Input: part model. Units: mm. Frame: model coordinates. Face numbers are marked on the shaded views. A direction names the side the tool comes from. Give positions to 0.01 mm unless a question says otherwise; leave off trailing zeros. Loops run counter-clockwise (first coordinate to the right, second up) from the corner with the lowest first, then second, coordinate; pieces in that order, holes last. Notation, with made-up numbers: (-34, -23.75) -> (3, -23.75) arc R6 ccw to (3, -15.75) -> close; hole circle Ø9 at (-29, -39). An arc over 180 degrees is marked (long way). Use CSV: the item, a comma, the result in double quotes.
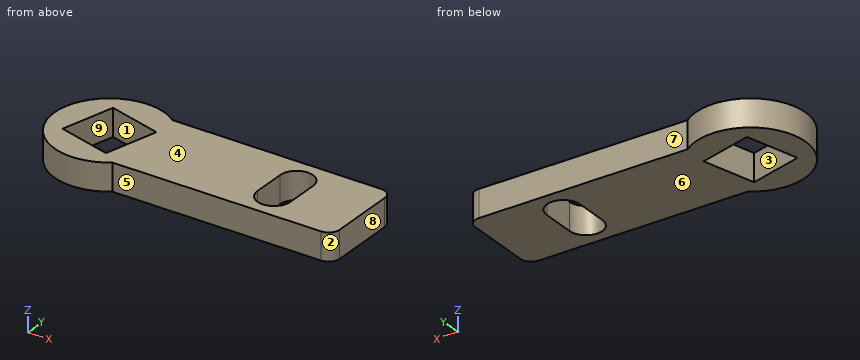
```python
from build123d import *

# Parameters (mm, degrees)
EXTRUDE_1_DEPTH     = 1.25
CUT_EXTRUDE_1_DEPTH = 24.669600757
FILLET_1_R          = 1


with BuildPart() as part:
    # 草图1 → 凸台-拉伸1 (new, symmetric)
    with BuildSketch(Plane.XY):
        with BuildLine():
            Line((3, 4), (23, 4))
            Line((23, 4), (23, -4))
            Line((23, -4), (3, -4))
            ThreePointArc((3, -4), (-5, 0), (3, 4))
        make_face()
    extrude(amount=EXTRUDE_1_DEPTH, both=True)

    # 草图2 → 切除-拉伸1 (cut, through all)
    with BuildSketch(Plane.XY.offset(1.25)):
        Polygon((1.767766953, -3.061862178), (3.061862178, 1.767766953), (-1.767766953, 3.061862178), (-3.061862178, -1.767766953), align=None)
        with BuildLine():
            Line((14.5, -1.5), (14.5, 1.5))
            ThreePointArc((14.5, 1.5), (16, 3), (17.5, 1.5))
            Line((17.5, 1.5), (17.5, -1.5))
            ThreePointArc((17.5, -1.5), (16, -3), (14.5, -1.5))
        make_face()
    extrude(amount=-CUT_EXTRUDE_1_DEPTH, mode=Mode.SUBTRACT)

    # 圆角1
    fillet_1_edges = [part.edges().sort_by_distance(p)[0] for p in [
        (23, 4, 0),
        (23, -4, 0),
    ]]
    fillet(fillet_1_edges, radius=FILLET_1_R)


solid = part.part
```
1) Section query B-B (z = 0). Return loops of the section in (x, y).
From the geometry:
outline,"(3, -4) -> (22, -4) arc R1 ccw to (23, -3) -> (23, 3) arc R1 ccw to (22, 4) -> (3, 4) arc R5 ccw (long way) to start; hole (-3.06, -1.77) -> (1.77, -3.06) -> (3.06, 1.77) -> (-1.77, 3.06) -> close; hole (14.5, -1.5) arc R1.5 ccw to (17.5, -1.5) -> (17.5, 1.5) arc R1.5 ccw to (14.5, 1.5) -> close"
2) Mould query, pull axis Y, two halves, no side actions, for the marked faces 1, 2, 3 and 4. Classes: pulls with the +Y half, pulls with the -Y half, needs draft (parallel to the pull), parting line crosses it, or undercut.
From the geometry:
face 1,"undercut"
face 2,"pulls with the -Y half"
face 3,"undercut"
face 4,"needs draft"
3) Reachability of the marked faces 5, 6, 7, 8 and 9 from +Z, -Z, +X, -X, +Y, -Y: full face, straight path, thin tool, end or side. Return the list, or none.
From the geometry:
face 5,"+Z, -Z, +X, -Y"
face 6,"-Z, +X, -X, +Y, -Y"
face 7,"+Z, -Z, +X, +Y"
face 8,"+Z, -Z, +X, +Y, -Y"
face 9,"+Z, -Z"
4) Section query C-C (y = -2.5). Return loops of the section in (x, z), then the cut area to 3 significant figures.
From the geometry:
outline,"(-4.33, -1.25) -> (-0.33, -1.25) -> (-0.33, 1.25) -> (-4.33, 1.25) -> close; (1.92, -1.25) -> (14.88, -1.25) -> (14.88, 1.25) -> (1.92, 1.25) -> close; (17.12, -1.25) -> (23, -1.25) -> (23, 1.25) -> (17.12, 1.25) -> close"
area,"57.1 mm^2"
5) Ray query, line 1 (X direction, y = 1, z = -0.3); line 2 (X direction, y = 0.25, z = 0.55); line 3 (Y direction, x = 8.25, z = 0.4). Return the intervals inside material, ascending.
From the geometry:
line 1,"x = -4.9 to -2.32, 2.86 to 14.5, 17.5 to 23"
line 2,"x = -4.99 to -2.52, 2.66 to 14.5, 17.5 to 23"
line 3,"y = -4 to 4"
6) Section query D-D (x = 0). Return loops of the section in (y, z).
From the geometry:
outline,"(-5, -1.25) -> (-2.59, -1.25) -> (-2.59, 1.25) -> (-5, 1.25) -> close; (2.59, -1.25) -> (5, -1.25) -> (5, 1.25) -> (2.59, 1.25) -> close"
7) Contact query for a flat-ended pin moving along its axis: pin 1 (1 mm diameter, centred on y = 3.5, z = 0.5, fed in from -X). Output: stop coordinate, or through.
From the geometry:
pin 1,"stops at x = -4"
8) Section query A-A (x = 16). Return loops of the section in (y, z), then the cut area to 3 significant figures.
From the geometry:
outline,"(-4, -1.25) -> (-3, -1.25) -> (-3, 1.25) -> (-4, 1.25) -> close; (3, -1.25) -> (4, -1.25) -> (4, 1.25) -> (3, 1.25) -> close"
area,"5.00 mm^2"
